The model under review builds one solid part; all positions refer to its coordinate system, in mm. Coordinates: 2 decimals unless noted, no trailing zeros. Write each loop counter-clockwise with the first axis right and the second up, starting at its lowest first coordinate (ties: lowest second). Pieces come first, ordered by that corner, then holes. Notation, with made-up numbers: (67.25, 23) - (124.25, 23) arc R6 ccw to (124.25, 34) - close; hole circle Ø1 at (14, -13). An arc over 180 degrees is marked (long way). Put each result on its own line as item: value.
from build123d import *

# Parameters (mm, degrees)
HEX_PROFILE_SKETCH_R = 6
HEX_NUT_BODY_DEPTH   = 5


with BuildPart() as part:
    # Hex Profile Sketch → Hex Nut Body (new, symmetric)
    with BuildSketch(Plane(origin=(0, 0, 0), x_dir=(1, 0, 0), z_dir=(0, 1, 0))):
        Polygon((13.856406461, 0), (6.92820323, 12), (-6.92820323, 12), (-13.856406461, 0), (-6.92820323, -12), (6.92820323, -12), align=None)
        with Locations(Location((0, 0, 0), (0, 0, 270))):
            Circle(HEX_PROFILE_SKETCH_R, mode=Mode.SUBTRACT)
    extrude(amount=HEX_NUT_BODY_DEPTH, both=True)

    # Corner Chamfer Profile Sketch → Hex Corner Chamfer (revolve, cut)
    with BuildSketch(Plane.XY, mode=Mode.PRIVATE) as hex_corner_chamfer_sk:
        with BuildLine():
            Line((11.856406461, 5), (13.856406461, 5))
            Line((13.856406461, 5), (13.856406461, 3))
            ThreePointArc((13.856406461, 3), (13.106898111, 4.25049165), (11.856406461, 5))
        make_face()
    revolve(hex_corner_chamfer_sk.sketch.rotate(Axis((0, -7.51909737, 0), (0, 1, 0)), 90), axis=Axis((0, -7.51909737, 0), (0, 1, 0)), mode=Mode.SUBTRACT)


solid = part.part
1. The part is to be moulded in two halves that separate along Z. For faces 1 (the flat face through (0, 0, 12)), 2 (the flat face through (3, -5, -6)), 3 (the cylindrical face through (1.802, -0.07, 5.723)), say which applies: +Z half, -Z half, draft (parallel to the pull), parting line (faces both ways), or undercut.
Determined:
face 1: +Z half
face 2: draft
face 3: undercut
2. For pin 1 Ø1 at (y, z) = (0, 2) entering from -X; pin 2 Ø3 at (y, z) = (3.5, -8) entering from -X, all flat-tipped, find the tip position at first contact; note any pin that passes through.
Determined:
pin 1: stops at x = -12.99
pin 2: stops at x = -10.1
3. Consider section B-B on y = 2.5. State the section outline as (x, z) points, plus the area to 3 significant figures.
Determined:
outline: (-13.86, 0) - (-6.93, -12) - (6.93, -12) - (13.86, 0) - (6.93, 12) - (-6.93, 12) - close; hole circle Ø12 at (0, 0)
area: 386 mm^2
4. Consider section C-C on y = 4. State the section outline as (x, z) points.
Determined:
outline: (-13.3, -0.97) - (-7.49, -11.03) arc R13.33 ccw to (-5.81, -12) - (5.81, -12) arc R13.33 ccw to (7.49, -11.03) - (13.3, -0.97) arc R13.33 ccw to (13.3, 0.97) - (7.49, 11.03) arc R13.33 ccw to (5.81, 12) - (-5.81, 12) arc R13.33 ccw to (-7.49, 11.03) - (-13.3, 0.97) arc R13.33 ccw to start; hole circle Ø12 at (0, 0)
5. To check wall thickness, follow probe 1 along X at (y, z) = (4.5, -1); probe 2 along Z at (x, y) = (-5.25, -2.5); probe 3 along X at (y, z) = (2.75, -4.75). State the ranges of each line that lie inside material, in increasing order.
Determined:
probe 1: x = -12.78 to -5.92, 5.92 to 12.78
probe 2: z = -12 to -2.9, 2.9 to 12
probe 3: x = -11.11 to -3.67, 3.67 to 11.11
6. Consider section A-A on x = 0. State the section outline as (y, z) points.
Determined:
outline: (-5, -12) - (4.95, -12) arc R3 ccw to (5, -11.86) - (5, -6) - (-5, -6) - close; (-5, 6) - (5, 6) - (5, 11.86) arc R3 ccw to (4.95, 12) - (-5, 12) - close
